from build123d import *

# Parameters (mm, degrees)
M24_TAPPED_HOLE1_D     = 21
M24_TAPPED_HOLE1_DEPTH = 57
M24_TAPPED_HOLE1_TIP   = 6.3090365
SKETCH4_R              = 5
CUT_EXTRUDE1_DEPTH     = 25
FILLET2_R              = 2
FILLET3_R              = 4


with BuildPart() as part:
    # Sketch1 → Revolve1 (revolve)
    with BuildSketch(Plane.XY, mode=Mode.PRIVATE) as revolve1_sk:
        with BuildLine():
            Line((67, 27.5), (67, 20))
            Line((67, 20), (0, 20))
            Line((0, 20), (0, 0))
            Line((0, 0), (77.589222534, 0))
            ThreePointArc((77.589222534, 0), (78.70107404, 12.20097289), (82, 24))
            Line((82, 24), (82, 27.5))
            Line((82, 27.5), (67, 27.5))
        make_face()
    revolve(revolve1_sk.sketch.rotate(Axis((0, 0, 0), (1, 0, 0)), 90), axis=Axis((0, 0, 0), (1, 0, 0)))

    # M24 Tapped Hole1
    with Locations(Plane.ZY):
        with Locations((0, 0)):
            Hole(M24_TAPPED_HOLE1_D / 2, depth=M24_TAPPED_HOLE1_DEPTH)
            with Locations((0, 0, -(M24_TAPPED_HOLE1_DEPTH + M24_TAPPED_HOLE1_TIP / 2))):  # 118° drill point
                Cone(0, M24_TAPPED_HOLE1_D / 2, M24_TAPPED_HOLE1_TIP, mode=Mode.SUBTRACT)

    # Sketch4 → Cut-Extrude1 (cut, symmetric)
    with BuildSketch(Plane(origin=(0, 0, 0), x_dir=(1, 0, 0), z_dir=(0, 1, 0))):
        with Locations(Location((35, 0, 0), (0, 0, 270))):
            Circle(SKETCH4_R)
    extrude(amount=CUT_EXTRUDE1_DEPTH, both=True, mode=Mode.SUBTRACT)

    # Fillet2
    fillet2_edges = [part.edges().sort_by_distance(p)[0] for p in [
        (82, 0, -27.5),
    ]]
    fillet(fillet2_edges, radius=FILLET2_R)

    # Fillet3
    fillet3_edges = [part.edges().sort_by_distance(p)[0] for p in [
        (67, 0, -27.5),
    ]]
    fillet(fillet3_edges, radius=FILLET3_R)


solid = part.part
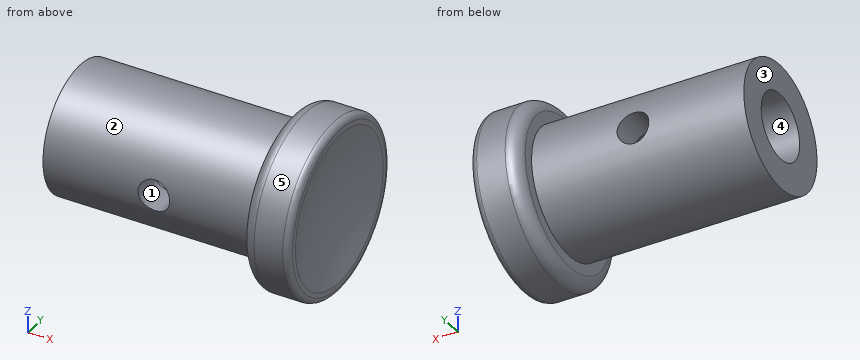
Design review of the part built by this model. Coordinates are the model's own, in mm. Face numbers are marked on the shaded views. A direction names the side the tool comes from. Round coordinates to 2 decimals unless told otherwise and drop trailing zeros. Write each loop counter-clockwise with the first axis right and the second up, starting at its lowest first coordinate (ties: lowest second). Pieces come first, ordered by that corner, then holes. Notation, with made-up numbers: (75, 25.25) - (91, 25.25) arc R21 ccw to (91, 60.25) - close; hole circle Ø10 at (41.25, -16.75). An arc over 180 degrees is marked (long way). Return JSON: item names as keys, results as strings. Group by question number.
Item 1: We need section B-B on x = 49. Write out the cut boundary in (y, z).
Item 2: We need section A-A on x = 35. Write out the cut boundary in (y, z).
Item 3: The part is to be moulded in two halves that separate along Z. For the marked faces 1, 2 and 3, say which applies: pulls with the +Z half, pulls with the -Z half, needs draft (parallel to the pull), parting line crosses it, or undercut.
Item 4: Machinability: for the marked faces 4 and 5, which of the approach directions +Z, -Z, +X, -X, +Y, -Y give a long, thin tool a straight path to every point of the face, cutting with its end or side? Answer none if there is none.
Item 5: Insertion check: P1, Ø12.5, axis at y = 0, z = 0, coming from the -X side; P2, Ø4, axis at y = -1.5, z = 1.5, coming from the -X side; P3, Ø6, axis at x = 35, z = 0, coming from the -Y side; P4, Ø5, axis at x = 63, z = -11, coming from the -Y side. Each pin has a flat end and moves straight along its axis. Give the tip position at first contact, or say it passes through.
Item 6: For probe 1 along X at (y, z) = (-11, 0); probe 2 along Y at (x, z) = (54, 1); probe 3 along X at (y, z) = (-16, 8), list the stretches that pass through material, from the lowest coordinate up. Write a range as [from, to].
Item 7: We need section C-C on x = 75.5. Write out the cut boundary in (y, z).
Item 8: We need section D-D on x = 60. Write out the cut boundary in (y, z), and give its area (3 significant figures).
Model answer:
{
 "1": {"outline": "circle Ø40 at (0, 0); hole circle Ø21 at (0, 0)"},
 "2": {"outline": "(-19.36, -5) arc R20 ccw to (19.36, -5) - (9.23, -5) arc R10.5 cw to (-9.23, -5) - close; (-19.36, 5) - (-9.23, 5) arc R10.5 cw to (9.23, 5) - (19.36, 5) arc R20 ccw to start"},
 "3": {"face 1": "undercut", "face 2": "parting line crosses it", "face 3": "needs draft"},
 "4": {"face 4": "-X", "face 5": "+X, -X"},
 "5": {"P1": "stops at x = 59.55", "P2": "stops at x = 60.83", "P3": "passes through", "P4": "stops at y = -18.1"},
 "6": {"probe 1": "x = [0, 30], [40, 78.49]", "probe 2": "y = [-19.97, -10.45], [10.45, 19.97]", "probe 3": "x = [0, 80]"},
 "7": {"outline": "circle Ø55 at (0, 0)"},
 "8": {"outline": "circle Ø40 at (0, 0); hole circle Ø11.01 at (0, 0)", "area": "1,160 mm²"}
}
